```python
from build123d import *

# Parameters (mm, degrees)
SKETCH1_R           = 9
SKETCH1_R_2         = 4.5
BOSS_EXTRUDE1_DEPTH = 10
SKETCH2_R           = 85
BOSS_EXTRUDE2_DEPTH = 60
SKETCH3_R           = 71
CUT_EXTRUDE1_DEPTH  = 60
FILLET1_R           = 1.5
SCALE1_SCALE        = 0.5
SKETCH_1_R          = 2.25
EXTRUDE_1_DEPTH     = 5
SKETCH_2_R          = 4
CUT_EXTRUDE_1_DEPTH = 10


with BuildPart() as part:
    # Sketch1 → Boss-Extrude1 (new body)
    with BuildSketch(Plane.XY):
        with BuildLine():
            Line((-81, -90), (81, -90))
            ThreePointArc((81, -90), (87.363961031, -87.363961031), (90, -81))
            Line((90, -81), (90, 81))
            ThreePointArc((90, 81), (87.363961031, 87.363961031), (81, 90))
            Line((81, 90), (-81, 90))
            ThreePointArc((-81, 90), (-87.363961031, 87.363961031), (-90, 81))
            Line((-90, 81), (-90, -81))
            ThreePointArc((-90, -81), (-87.363961031, -87.363961031), (-81, -90))
        make_face()
        Circle(SKETCH1_R, mode=Mode.SUBTRACT)
        with Locations((70, 70)):
            Circle(SKETCH1_R_2, mode=Mode.SUBTRACT)
        with Locations(Location((-70, 70, 0), (0, 0, 180))):
            Circle(SKETCH1_R_2, mode=Mode.SUBTRACT)
        with Locations(Location((70, -70, 0), (0, 0, 180))):
            Circle(SKETCH1_R_2, mode=Mode.SUBTRACT)
        with Locations((-70, -70)):
            Circle(SKETCH1_R_2, mode=Mode.SUBTRACT)
    extrude(amount=BOSS_EXTRUDE1_DEPTH)

    # Sketch2 → Boss-Extrude2 (add)
    with BuildSketch(Plane.XY.offset(10)):
        with Locations(Location((0, 0, 0), (0, 0, 180))):
            Circle(SKETCH2_R)
    extrude(amount=BOSS_EXTRUDE2_DEPTH)

    # Sketch3 → Cut-Extrude1 (cut)
    with BuildSketch(Plane.XY.offset(70)):
        Circle(SKETCH3_R)
    extrude(amount=-CUT_EXTRUDE1_DEPTH, mode=Mode.SUBTRACT)

    # Fillet1
    fillet1_edges = [part.edges().sort_by_distance(p)[0] for p in [
        (87.363961031, 87.363961031, 10),
        (0, 90, 10),
        (-87.363961031, 87.363961031, 10),
        (-90, 0, 10),
        (-87.363961031, -87.363961031, 10),
        (0, -90, 10),
        (87.363961031, -87.363961031, 10),
        (85, 0, 10),
        (85, 0, 70),
        (-71, 0, 10),
        (90, 0, 10),
    ]]
    fillet(fillet1_edges, radius=FILLET1_R)


with BuildPart() as part_1:
    # Scale1: scaled about (0, 0, 0)
    add(part.part.scale(SCALE1_SCALE))

    # 草图1 → 凸台-拉伸1 (add)
    with BuildSketch(Plane(origin=(0, 0, 0), x_dir=(-1, 0, 0), z_dir=(0, 0, -1))):
        with Locations((35, -35)):
            Circle(SKETCH_1_R)
        with Locations((-35, -35)):
            Circle(SKETCH_1_R)
        with Locations((-35, 35)):
            Circle(SKETCH_1_R)
        with Locations((35, 35)):
            Circle(SKETCH_1_R)
    extrude(amount=-EXTRUDE_1_DEPTH)

    # 草图2 → 切除-拉伸1 (cut)
    with BuildSketch(Plane(origin=(0, 0, 0), x_dir=(-1, 0, 0), z_dir=(0, 0, -1))):
        with Locations((-37.5, 37.5)):
            Circle(SKETCH_2_R)
        with Locations(Location((-37.5, -37.5, 0), (0, 0, 180))):
            Circle(SKETCH_2_R)
        with Locations(Location((37.5, 37.5, 0), (0, 0, 180))):
            Circle(SKETCH_2_R)
        with Locations((37.5, -37.5)):
            Circle(SKETCH_2_R)
    extrude(amount=-CUT_EXTRUDE_1_DEPTH, mode=Mode.SUBTRACT)


solid = part_1.part
```
Geometry: final body of the model. Coordinates: model frame, mm. A direction names the side the tool comes from. Give positions to 0.01 mm unless a question says otherwise; leave off trailing zeros. Write each loop counter-clockwise with the first axis right and the second up, starting at its lowest first coordinate (ties: lowest second). Pieces come first, ordered by that corner, then holes.
1. Section query C-C, the plane z = 8. Return loops of the section in (x, y).
2. Draft query along Y for faces 1 (the cylindrical face through (-43.647, 43.717, 2.095)), 2 (the cylindrical face through (-38.021, 33.534, 2.465)), 3 (the flat face through (1, 11, 0)), 4 (the cylindrical face through (38.021, 41.466, 2.465)). Return one class per face: released by +Y, released by -Y, zero draft, split by the parting line, or undercut.
3. Pin query (flat end, axial travel): P1, Ø11.5, axis at x = 0, y = 0, coming from the +Z side; P2, Ø8, axis at x = 0.5, z = 25.5, coming from the +Y side; P3, Ø10, axis at x = -3.5, z = 18.5, coming from the -Y side; P4, Ø13, axis at x = -37.5, y = -37.5, coming from the -Z side. Return the tip coordinate at first contact, or that it passes through.
4. Section query A-A, the plane y = 0. Return loops of the section in (x, z).
5. Reachability of faces 5 (the cylindrical face through (43.647, -43.717, 2.095)), 6 (the cylindrical face through (-40.537, -12.766, 19.8)) from +Z, -Z, +X, -X, +Y, -Y: full face, straight path, thin tool, end or side. Return the list, or none.
6. Section query D-D, the plane x = -37.5. Count the separate pieces of the cut face and the enclosed holes in it, then the cut area to 3 significant figures.
7. Line query: probe 1 along Y at (x, z) = (-37.5, 3.1); probe 2 along Y at (x, z) = (0, 28); probe 3 along Z at (x, y) = (-20, -39). Output: solid intervals per line, ascending.
Computed:
1. outline: circle Ø85 at (0, 0); hole circle Ø71 at (0, 0)
2. face 1: released by +Y
2. face 2: undercut
2. face 3: zero draft
2. face 4: undercut
3. P1: stops at z = 5
3. P2: stops at y = 42.5
3. P3: stops at y = -42.5
3. P4: stops at z = 0
4. outline: (-45, 0) - (-4.5, 0) - (-4.5, 5) - (-34.75, 5) arc R0.75 cw to (-35.5, 5.75) - (-35.5, 35) - (-41.75, 35) arc R0.75 ccw to (-42.5, 34.25) - (-42.5, 5.75) arc R0.75 cw to (-43.25, 5) - (-44.25, 5) arc R0.75 ccw to (-45, 4.25) - close; (4.5, 0) - (45, 0) - (45, 4.25) arc R0.75 ccw to (44.25, 5) - (43.25, 5) arc R0.75 cw to (42.5, 5.75) - (42.5, 34.25) arc R0.75 ccw to (41.75, 35) - (35.5, 35) - (35.5, 5.75) arc R0.75 cw to (34.75, 5) - (4.5, 5) - close
5. face 5: +Z, -Z, +X, -Y
5. face 6: +Z
6. separate pieces: 3
6. enclosed holes: 0
6. area: 1,570 mm2
7. probe 1: y = -45 to -41.5, -33.5 to 33.5, 41.5 to 45
7. probe 2: y = -42.5 to -35.5, 35.5 to 42.5
7. probe 3: z = 0 to 5
